from build123d import *
from build123d.topology import SkipClean

# Parameters (mm, degrees)
BASE_PLATE_DEPTH                = 15
CIRCULAR_START                  = 35
CIRCULAR_HOUSING_DEPTH          = 35
HOUSING_EXTENSION_SKETCH_R      = 65
HOUSING_EXTENSION_SKETCH_R_2    = 25
HOUSING_EXTENSION_DEPTH         = 15
CLEVIS_LUG_BLOCK_SKETCH_R       = 25
CLEVIS_LUG_BLOCK_SKETCH_R_2     = 10
CLEVIS_LUG_BLOCK_DEPTH          = 30
CLEVIS_START                    = -30
CLEVIS_LUG_EXTENSION_SKETCH_R   = 25
CLEVIS_LUG_EXTENSION_SKETCH_R_2 = 10
CLEVIS_LUG_EXTENSION_DEPTH      = 30
PIVOT_LUG_SKETCH_R              = 25
PIVOT_LUGS_DEPTH                = 30
PIVOT_PIN_HOLE_SKETCH_R         = 10
PIVOT_PIN_HOLE_20_DEPTH         = 200
CLEVIS_SLOT_25_DEPTH            = 200
SPOT_FACE_A_SKETCH_R            = 18
SPOT_FACE_A_36X5_DEPTH          = 5
LUG_START                       = -30
LUG_FILL_BOSS_DEPTH             = 30
SPOT_START                      = -5
SPOT_FACE_B_SKETCH_R            = 18
SPOT_FACE_B_36X5_DEPTH          = 5


with BuildPart() as part:
    # Base Plate Sketch → Base Plate (new body)
    with BuildSketch(Plane(origin=(0, 0, 0), x_dir=(1, 0, 0), z_dir=(0, 1, 0))):
        with BuildLine():
            ThreePointArc((64.226162893, -10), (0, -65), (-64.226162893, -10))
            Line((-64.226162893, -10), (-79.372539332, -10))
            ThreePointArc((-79.372539332, -10), (-52.915026221, -60), (0, -80))
            ThreePointArc((0, -80), (52.915026221, -60), (79.372539332, -10))
            Line((79.372539332, -10), (64.226162893, -10))
        make_face()
        with BuildLine():
            ThreePointArc((0, 80), (-52.915026221, 60), (-79.372539332, 10))
            Line((-79.372539332, 10), (-64.226162893, 10))
            ThreePointArc((-64.226162893, 10), (0, 65), (64.226162893, 10))
            Line((64.226162893, 10), (79.372539332, 10))
            ThreePointArc((79.372539332, 10), (52.915026221, 60), (0, 80))
        make_face()
        with BuildLine():
            Line((200, 80), (0, 80))
            ThreePointArc((0, 80), (52.915026221, 60), (79.372539332, 10))
            Line((79.372539332, 10), (100, 10))
            Line((100, 10), (100, 50))
            Line((100, 50), (200, 50))
            Line((200, 50), (200, 80))
        make_face()
        with BuildLine():
            ThreePointArc((79.372539332, -10), (52.915026221, -60), (0, -80))
            Line((0, -80), (200, -80))
            Line((200, -80), (200, -50))
            Line((200, -50), (100, -50))
            Line((100, -50), (100, -10))
            Line((100, -10), (79.372539332, -10))
        make_face()
    extrude(amount=BASE_PLATE_DEPTH)

    # Circular Housing Sketch → Circular Housing (add)
    with BuildSketch(Plane.XZ.offset(CIRCULAR_START)):
        with BuildLine():
            ThreePointArc((79.372539332, 10), (52.915026221, 60), (0, 80))
            ThreePointArc((0, 80), (-52.915026221, 60), (-79.372539332, 10))
            Line((-79.372539332, 10), (-64.226162893, 10))
            ThreePointArc((-64.226162893, 10), (0, 65), (64.226162893, 10))
            Line((64.226162893, 10), (79.372539332, 10))
        make_face()
        with BuildLine():
            Line((-64.226162893, 10), (-79.372539332, 10))
            ThreePointArc((-79.372539332, 10), (-60, -52.915026221), (0, -80))
            ThreePointArc((0, -80), (56.568542495, -56.568542495), (80, 0))
            ThreePointArc((80, 0), (79.842980739, 5.009833003), (79.372539332, 10))
            Line((79.372539332, 10), (64.226162893, 10))
            ThreePointArc((64.226162893, 10), (64.806251967, 5.014948252), (65, 0))
            ThreePointArc((65, 0), (-5.014948252, -64.806251967), (-64.226162893, 10))
        make_face()
        with BuildLine():
            Line((200, 80), (0, 80))
            ThreePointArc((0, 80), (52.915026221, 60), (79.372539332, 10))
            Line((79.372539332, 10), (100, 10))
            Line((100, 10), (100, 50))
            Line((100, 50), (200, 50))
            Line((200, 50), (200, 80))
        make_face()
        with BuildLine():
            Line((100, 10), (79.372539332, 10))
            ThreePointArc((79.372539332, 10), (79.842980739, 5.009833003), (80, 0))
            ThreePointArc((80, 0), (56.568542495, -56.568542495), (0, -80))
            Line((0, -80), (200, -80))
            Line((200, -80), (200, -50))
            Line((200, -50), (100, -50))
            Line((100, -50), (100, 10))
        make_face()
    extrude(amount=-CIRCULAR_HOUSING_DEPTH)

    # Housing Extension Sketch → Housing Extension (add)
    with BuildSketch(Plane.XZ.offset(35)):
        with Locations(Location((0, 0, 0), (0, 0, 270))):
            Circle(HOUSING_EXTENSION_SKETCH_R)
        with Locations(Location((0, 0, 0), (0, 0, 270))):
            Circle(HOUSING_EXTENSION_SKETCH_R_2, mode=Mode.SUBTRACT)
    extrude(amount=-HOUSING_EXTENSION_DEPTH)

    # Clevis Lug Block Sketch → Clevis Lug Block (add)
    # profile 1 of 2: a face of its own
    with SkipClean():  # the faces are left unmerged after this step: merging them gives an invalid solid
        with BuildSketch(Plane.XY.offset(80)):
            with BuildLine():
                Line((75, -35), (75, -71.5))
                ThreePointArc((75, -71.5), (100, -46.5), (125, -71.5))
                Line((125, -71.5), (125, -35))
                Line((125, -35), (75, -35))
            make_face()
        # profile 2 of 2: a face of its own
        with BuildSketch(Plane.XY.offset(80)):
            with Locations((100, -71.5)):
                Circle(CLEVIS_LUG_BLOCK_SKETCH_R)
            with Locations((100, -71.5)):
                Circle(CLEVIS_LUG_BLOCK_SKETCH_R_2, mode=Mode.SUBTRACT)
        extrude(amount=-CLEVIS_LUG_BLOCK_DEPTH)

    # Clevis Lug Extension Sketch → Clevis Lug Extension (add)
    # profile 1 of 2: a face of its own
    with SkipClean():  # the faces are left unmerged after this step: merging them gives an invalid solid
        with BuildSketch(Plane(origin=(0, 0, -80), x_dir=(-1, 0, 0), z_dir=(0, 0, -1)).offset(CLEVIS_START)):
            with BuildLine():
                Line((-125, -35), (-125, -71.5))
                ThreePointArc((-125, -71.5), (-100, -46.5), (-75, -71.5))
                Line((-75, -71.5), (-75, -35))
                Line((-75, -35), (-125, -35))
            make_face()
        # profile 2 of 2: a face of its own
        with BuildSketch(Plane(origin=(0, 0, -80), x_dir=(-1, 0, 0), z_dir=(0, 0, -1)).offset(CLEVIS_START)):
            with Locations((-100, -71.5)):
                Circle(CLEVIS_LUG_EXTENSION_SKETCH_R)
            with Locations(Location((-100, -71.5, 0), (0, 0, 180))):
                Circle(CLEVIS_LUG_EXTENSION_SKETCH_R_2, mode=Mode.SUBTRACT)
        extrude(amount=CLEVIS_LUG_EXTENSION_DEPTH)

    # Pivot Lug Sketch → Pivot Lugs (add)
    with SkipClean():  # the faces are left unmerged after this step: merging them gives an invalid solid
        with BuildSketch(Plane.XY.offset(80)):
            with Locations((200, -10)):
                Circle(PIVOT_LUG_SKETCH_R)
        extrude(amount=-PIVOT_LUGS_DEPTH)

    # Pivot Pin Hole Sketch → Pivot Pin Hole _20 (cut)
    with SkipClean():  # the faces are left unmerged after this step: merging them gives an invalid solid
        with BuildSketch(Plane.XY.offset(80)):
            with Locations((200, -10)):
                Circle(PIVOT_PIN_HOLE_SKETCH_R)
        extrude(amount=-PIVOT_PIN_HOLE_20_DEPTH, mode=Mode.SUBTRACT)

    # Clevis Slot Sketch → Clevis Slot 25 (cut)
    with SkipClean():  # the faces are left unmerged after this step: merging them gives an invalid solid
        with BuildSketch(Plane.XY.offset(80)):
            with BuildLine():
                Line((200, 15), (200, -10))
                Line((200, -10), (225, -10))
                ThreePointArc((225, -10), (217.67766953, 7.67766953), (200, 15))
            make_face()
        extrude(amount=-CLEVIS_SLOT_25_DEPTH, mode=Mode.SUBTRACT)

    # Spot Face A Sketch → Spot Face A _36x5 (cut)
    with SkipClean():  # the faces are left unmerged after this step: merging them gives an invalid solid
        with BuildSketch(Plane.XY.offset(80)):
            with Locations((200, -10)):
                Circle(SPOT_FACE_A_SKETCH_R)
        extrude(amount=-SPOT_FACE_A_36X5_DEPTH, mode=Mode.SUBTRACT)

    # Lug Fill Sketch → Lug Fill Boss (add)
    with SkipClean():  # the faces are left unmerged after this step: merging them gives an invalid solid
        with BuildSketch(Plane(origin=(0, 0, -80), x_dir=(-1, 0, 0), z_dir=(0, 0, -1)).offset(LUG_START)):
            with BuildLine():
                Line((-210, -10), (-225, -10))
                ThreePointArc((-225, -10), (-217.67766953, -27.67766953), (-200, -35))
                Line((-200, -35), (-200, -20))
                ThreePointArc((-200, -20), (-207.071067812, -17.071067812), (-210, -10))
            make_face()
        extrude(amount=LUG_FILL_BOSS_DEPTH)

    # Spot Face B Sketch → Spot Face B _36x5 (cut)
    with SkipClean():  # the faces are left unmerged after this step: merging them gives an invalid solid
        with BuildSketch(Plane(origin=(0, 0, -80), x_dir=(-1, 0, 0), z_dir=(0, 0, -1)).offset(SPOT_START)):
            with Locations((-200, -10)):
                Circle(SPOT_FACE_B_SKETCH_R)
        extrude(amount=SPOT_FACE_B_36X5_DEPTH, mode=Mode.SUBTRACT)


solid = part.part
Could you check a few things on this model? Use its own coordinates, in mm. A direction names the side the tool comes from. Give positions to 0.01 mm unless a question says otherwise; leave off trailing zeros. Order: outer loops, then holes, each group sorted by start corner. A loop starts at its lowest first (then second) coordinate and runs counter-clockwise, first axis right, second up.
1. For pin 1 (12 mm diameter, centred on x = 215, z = 66, fed in from +Y); pin 2 (16.5 mm diameter, centred on x = -70.5, y = 4, fed in from -Z); pin 3 (8 mm diameter, centred on x = -12.5, z = 29, fed in from -Y), each with a flat end and sliding along its axis, tell me the tip position at first contact or that it passes through.
Answers below:
pin 1: stops at y = -10
pin 2: stops at z = -50.25
pin 3: stops at y = -35
2. Suppose I cut it at D-D (z = 31). Write out the boundary of the cut face in (x, y), plus the area to 3 significant figures.
Answers below:
outline: (-73.75, -35) - (100, -35) - (100, 15) - (57.13, 15) - (57.13, -20) - (-57.13, -20) - (-57.13, 15) - (-73.75, 15) - close
area: 4,690 mm2
3. Suppose I cut it at A-A (y = -58). Write out the boundary of the cut face in (x, z), plus the area to 3 significant figures.
Answers below:
outline: (75, -80) - (125, -80) - (125, -50) - (75, -50) - close; (75, 50) - (125, 50) - (125, 80) - (75, 80) - close
area: 3,000 mm2
4. Thinking about a two-plate mould opening in Y: for faces 1 (the cylindrical face through (92.63, -78.26, -64.79)), 2 (the flat face through (217, -10, -65)), 3 (the flat face through (125, -54, 65)), 4 (the cylindrical face through (217.871, -27.482, -64.79)), which applies, +Y half, -Y half, draft (parallel to the pull), parting line (faces both ways), or undercut?
Answers below:
face 1: undercut
face 2: +Y half
face 3: draft
face 4: -Y half
5. Which directions (+Z, -Z, +X, -X, +Y, -Y) give clear straight access to the entire face, cutting with the end or side of a thin tool? Please do faces 5 (the flat face through (82, 0, 0)), 6 (the flat face through (132, -29, 50)), 7 (the flat face through (1, -20, -28)), 8 (the flat face through (200, 7, -65)).
Answers below:
face 5: +X, -X, +Y
face 6: +X, -Y
face 7: +Y
face 8: +Z, -Z, +X, +Y
6. Suppose I cut it at B-B (y = -13.5). Write out the boundary of the cut face in (x, z), plus the area to 3 significant figures.
Answers below:
outline: (0, -80) - (182.34, -80) - (182.34, -75) - (190.63, -75) - (190.63, -50) - (100, -50) - (100, 50) - (190.63, 50) - (190.63, 75) - (182.34, 75) - (182.34, 80) - (0, 80) arc R80 ccw to start; (209.37, -75) - (217.66, -75) - (217.66, -80) - (224.75, -80) - (224.75, -50) - (209.37, -50) - close; (209.37, 50) - (224.75, 50) - (224.75, 80) - (217.66, 80) - (217.66, 75) - (209.37, 75) - close; hole circle Ø130 at (0, 0)
area: 19,000 mm2
7. Suppose I cut it at C-C (x = 11). Write out the boundary of the cut face in (y, z).
Answers below:
outline: (-35, -80) - (15, -80) - (15, -64.06) - (-20, -64.06) - (-20, -22.45) - (-35, -22.45) - close; (-35, 22.45) - (-20, 22.45) - (-20, 64.06) - (15, 64.06) - (15, 80) - (-35, 80) - close
8. I need wall thicknesses on L1, parallel to X at y = -71, z = 66; L2, parallel to X at y = -24.5, z = 0; L3, parallel to Y at x = 199, z = -57. Which ranges of each line are inside material? Lowest first, please.
Answers below:
L1: x = 75 to 90.01, 109.99 to 125
L2: x = -80 to -25, 25 to 100
L3: y = -35 to -19.95, -0.05 to 15
